Geometry: final body of the model. Coordinates: model frame, mm. Face numbers are marked on the shaded views. A direction names the side the tool comes from. Give positions to 0.01 mm unless a question says otherwise; leave off trailing zeros. Write each loop counter-clockwise with the first axis right and the second up, starting at its lowest first coordinate (ties: lowest second). Pieces come first, ordered by that corner, then holes.
Q1. Section A-A (y = -0.5). Return the cut outline in (x, z), plus the area to 3 significant figures.
Q2. Section D-D (y = 3.25). Return the cut outline in (x, z), plus the area to 3 significant figures.
Q3. Mould query, pull axis Y, two halves, no side actions, for the marked faces 1, 2, 3 and 4. Classes: +Y half, -Y half, draft (parallel to the pull), parting line (faces both ways), or undercut.
Q4. Pin query (flat end, axial travel): pin 1 Ø6.5 at (y, z) = (-0.5, 20) entering from +X; pin 2 Ø8 at (y, z) = (-2, -22) entering from +X. Return the tip coordinate at first contact, or that it passes through.
Q5. Line query: line 1 (Y direction, x = 7.5, z = 0); line 2 (Z direction, x = 6, y = -1.75); line 3 (Z direction, x = 9.5, y = -4). Output: solid intervals per line, ascending.
Q6. Reachability of the marked faces 5 and 6 from +Z, -Z, +X, -X, +Y, -Y: full face, straight path, thin tool, end or side. Return the list, or none.
Q7. Section C-C (x = 4.5). Return the cut outline in (y, z).
Q8. Section B-B (z = 0). Return the cut outline in (x, y).
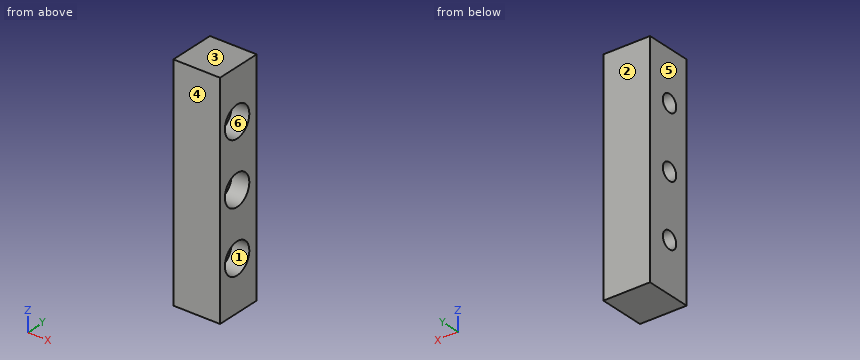
from build123d import *

# Parameters (mm, degrees)
SKETCH_1_W                = 72
SKETCH_1_H                = 15
EXTRUDE_1_DEPTH           = 15
HOLE_WIZARD_2_D           = 5.5
HOLE_WIZARD_2_CBORE_D     = 10
HOLE_WIZARD_2_CBORE_DEPTH = 5.7


with BuildPart() as part:
    # 草图1 → 凸台-拉伸1 (new body)
    with BuildSketch(Plane(origin=(0, 0, 0), x_dir=(0, 0, -1), z_dir=(1, 0, 0))):
        Rectangle(SKETCH_1_W, SKETCH_1_H)
    extrude(amount=EXTRUDE_1_DEPTH)

    # 打孔尺寸(%根据)内六角圆柱头螺钉的类型2 (through all)
    with Locations(Plane(origin=(15, 0, 0), x_dir=(0, 0, -1), z_dir=(1, 0, 0))):
        with Locations((-20, -0.5), (0, -0.5), (20, -0.5)):
            CounterBoreHole(HOLE_WIZARD_2_D / 2, HOLE_WIZARD_2_CBORE_D / 2, HOLE_WIZARD_2_CBORE_DEPTH)


solid = part.part
Computed:
1. outline: (0, -36) - (15, -36) - (15, -25) - (9.3, -25) - (9.3, -22.75) - (0, -22.75) - close; (0, -17.25) - (9.3, -17.25) - (9.3, -15) - (15, -15) - (15, -5) - (9.3, -5) - (9.3, -2.75) - (0, -2.75) - close; (0, 2.75) - (9.3, 2.75) - (9.3, 5) - (15, 5) - (15, 15) - (9.3, 15) - (9.3, 17.25) - (0, 17.25) - close; (0, 22.75) - (9.3, 22.75) - (9.3, 25) - (15, 25) - (15, 36) - (0, 36) - close
1. area: 756 mm2
2. outline: (0, -36) - (15, -36) - (15, -23.31) - (9.3, -23.31) - (9.3, -16.69) - (15, -16.69) - (15, -3.31) - (9.3, -3.31) - (9.3, 3.31) - (15, 3.31) - (15, 16.69) - (9.3, 16.69) - (9.3, 23.31) - (15, 23.31) - (15, 36) - (0, 36) - close
2. area: 967 mm2
3. face 1: undercut
3. face 2: +Y half
3. face 3: draft
3. face 4: -Y half
4. pin 1: stops at x = 9.3
4. pin 2: stops at x = 15
5. line 1: y = -7.5 to -3.25, 2.25 to 7.5
5. line 2: z = -36 to -22.45, -17.55 to -2.45, 2.45 to 17.55, 22.45 to 36
5. line 3: z = -36 to -23.57, -16.43 to -3.57, 3.57 to 16.43, 23.57 to 36
6. face 5: +Z, -Z, -X, +Y, -Y
6. face 6: +X
7. outline: (-7.5, -36) - (7.5, -36) - (7.5, 36) - (-7.5, 36) - close; hole circle Ø5.5 at (-0.5, -20); hole circle Ø5.5 at (-0.5, 0); hole circle Ø5.5 at (-0.5, 20)
8. outline: (0, -7.5) - (15, -7.5) - (15, -5.5) - (9.3, -5.5) - (9.3, -3.25) - (0, -3.25) - close; (0, 2.25) - (9.3, 2.25) - (9.3, 4.5) - (15, 4.5) - (15, 7.5) - (0, 7.5) - close
